Geometry check sheet. Reference: the model listing, model coordinates, mm. A direction names the side the tool comes from. Coordinates: 2 decimals unless noted, no trailing zeros. Loops run counter-clockwise (first coordinate to the right, second up) from the corner with the lowest first, then second, coordinate; pieces in that order, holes last.
from build123d import *

# Parameters (mm, degrees)
SLIDE_BLOCK_BODY_DEPTH       = 27.5
CENTRE_CHANNEL_37_WIDE_DEPTH = 20
TWIN_SLOTS_2XR6_DEPTH        = 38


with BuildPart() as part:
    # Block Profile Sketch → Slide Block Body (new, symmetric)
    with BuildSketch(Plane.XY):
        with BuildLine():
            Line((0, 0), (62.5, 0))
            Line((62.5, 0), (62.5, 10))
            Line((62.5, 10), (75, 10))
            ThreePointArc((75, 10), (65.627416998, 32.627416998), (43, 42))
            Line((43, 42), (0, 42))
            Line((0, 42), (-43, 42))
            ThreePointArc((-43, 42), (-65.627416998, 32.627416998), (-75, 10))
            Line((-75, 10), (-62.5, 10))
            Line((-62.5, 10), (-62.5, 0))
            Line((-62.5, 0), (0, 0))
        make_face()
    extrude(amount=SLIDE_BLOCK_BODY_DEPTH, both=True)

    # Centre Channel Sketch → Centre Channel 37 Wide (cut)
    with BuildSketch(Plane(origin=(0, 42, 0), x_dir=(1, 0, 0), z_dir=(0, 1, 0))):
        Polygon((0, 18.5), (92.62343554, 18.5), (92.62343554, -18.5), (-101.990097212, -18.5), (-101.990097212, 18.5), align=None)
    extrude(amount=-CENTRE_CHANNEL_37_WIDE_DEPTH, mode=Mode.SUBTRACT)

    # Twin Slots Sketch → Twin Slots 2xR6 (cut)
    with BuildSketch(Plane(origin=(0, 22, 0), x_dir=(1, 0, 0), z_dir=(0, 1, 0))):
        with BuildLine():
            Line((-14, -6), (-47, -6))
            ThreePointArc((-47, -6), (-53, 0), (-47, 6))
            Line((-47, 6), (-14, 6))
            ThreePointArc((-14, 6), (-8, 0), (-14, -6))
        make_face()
        with BuildLine():
            Line((14, 6), (47, 6))
            ThreePointArc((47, 6), (53, 0), (47, -6))
            Line((47, -6), (14, -6))
            ThreePointArc((14, -6), (8, 0), (14, 6))
        make_face()
    extrude(amount=-TWIN_SLOTS_2XR6_DEPTH, mode=Mode.SUBTRACT)


solid = part.part
(1) Access from +Z, -Z, +X, -X, +Y, -Y to the whole of each face (thin tool, end or side, straight path). Record for faces 1 (the flat face through (69, 10, 0)), 2 (the cylindrical face through (-8, 11, 0)), 3 (the flat face through (1, 32, -18.5)), 4 (the flat face through (-69, 10, 0)).
Findings:
face 1: +Z, -Z, +X, -Y
face 2: +Y, -Y
face 3: +X, -X, +Y
face 4: +Z, -Z, -X, -Y
(2) Sectioned sample at A-A on x = -19.5. Record the cut outline in (y, z).
Findings:
outline: (0, -27.5) - (42, -27.5) - (42, -18.5) - (22, -18.5) - (22, -6) - (0, -6) - close; (0, 6) - (22, 6) - (22, 18.5) - (42, 18.5) - (42, 27.5) - (0, 27.5) - close
(3) Sectioned sample at B-B on z = 0. Record the cut outline in (x, y).
Findings:
outline: (-75, 10) - (-62.5, 10) - (-62.5, 0) - (-53, 0) - (-53, 22) - (-72.66, 22) arc R32 ccw to start; (-8, 0) - (8, 0) - (8, 22) - (-8, 22) - close; (53, 0) - (62.5, 0) - (62.5, 10) - (75, 10) arc R32 ccw to (72.66, 22) - (53, 22) - close
(4) Draft check along X on faces 5 (the flat face through (-62.5, 5, 0)), 6 (the flat face through (1, 42, 23)), 7 (the flat face through (-31, 11, -6)), 8 (the flat face through (-30, 11, 6)). Enter one of: +X half, -X half, draft (parallel to the pull), parting line (faces both ways), or undercut.
Findings:
face 5: -X half
face 6: draft
face 7: undercut
face 8: undercut
(5) Sectioned sample at C-C on y = 37. Record the cut outline in (x, z), and give its area (3 significant figures).
Findings:
outline: (-60.18, -27.5) - (60.18, -27.5) - (60.18, -18.5) - (-60.18, -18.5) - close; (-60.18, 18.5) - (60.18, 18.5) - (60.18, 27.5) - (-60.18, 27.5) - close
area: 2,170 mm2
(6) Gauge pin test, flat ends, axial feed: pin 1 Ø4 at (y, z) = (23.5, -13) entering from -X; pin 2 Ø3 at (y, z) = (3, 6.5) entering from -X; pin 3 Ø4 at (x, z) = (-67, -11.5) entering from -Y. Record the tip position at first contact, or that the pin passes through.
Findings:
pin 1: stops at x = -72.86
pin 2: stops at x = -62.5
pin 3: stops at y = 10
(7) Sectioned sample at D-D on z = 20. Record the cut outline in (x, y), and give its area (3 significant figures).
Findings:
outline: (-75, 10) - (-62.5, 10) - (-62.5, 0) - (62.5, 0) - (62.5, 10) - (75, 10) arc R32 ccw to (43, 42) - (-43, 42) arc R32 ccw to start
area: 5,610 mm2
(8) Scan lines: L1, parallel to Z at x = 14.5, y = 24; L2, parallel to X at y = 8, z = 1.5; L3, parallel to X at y = 6.5, z = 5. Record each from-to range of solid material in increasing order.
Findings:
L1: z = -27.5 to -18.5, 18.5 to 27.5
L2: x = -62.5 to -52.81, -8.19 to 8.19, 52.81 to 62.5
L3: x = -62.5 to -50.32, -10.68 to 10.68, 50.32 to 62.5
